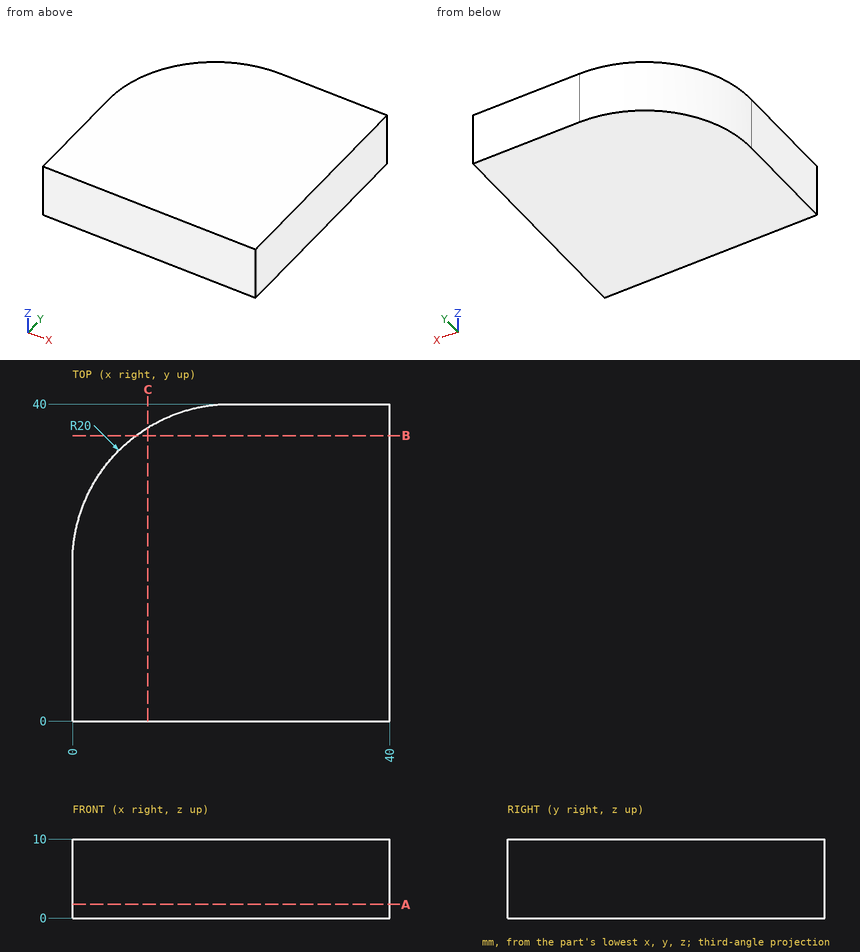
Geometry: see drawing. Coordinates: mm, zero at the bounding-box minimum. Round coordinates to 2 decimals unless told otherwise and drop trailing zeros. Write each loop counter-clockwise with the first axis right and the second up, starting at its lowest first coordinate (ties: lowest second). Pieces come first, ordered by that corner, then holes. Notation, with made-up numbers: M 85.5,7 L 100.5,7 A22 ccw 100.5,38 Z; hole C -6,37 d5. An arc over 180 degrees is marked long. Answer as a JSON object with one key per item and string values. Group by question number.
(1) Section query B-B on y = 36. Output: boundary loops of the cut face in (x, z), then the cut area to 3 significant figures.
(2) Section query C-C on x = 9.5. Output: boundary loops of the cut face in (y, z).
(3) Ray query, line 1 (X direction, y = 23.5, z = 2.75); line 2 (Y direction, x = 9.5, z = 5.25); line 3 (X direction, y = 36.5, z = 4.5). Return the intervals inside material, ascending. Write a range as [from, to].
(4) Section query A-A on z = 1.75. Output: boundary loops of the cut face in (x, y), then the cut area to 3 significant figures.
Computed values:
{
 "1": {"outline": "M 8,0 L 40,0 L 40,10 L 8,10 Z", "area": "320 mm^2"},
 "2": {"outline": "M 0,0 L 37.02,0 L 37.02,10 L 0,10 Z"},
 "3": {"line 1": "[0.31, 40]", "line 2": "[0, 37.02]", "line 3": "[8.7, 40]"},
 "4": {"outline": "M 0,0 L 40,0 L 40,40 L 20,40 A20 ccw 0,20 Z", "area": "1,510 mm^2"}
}
